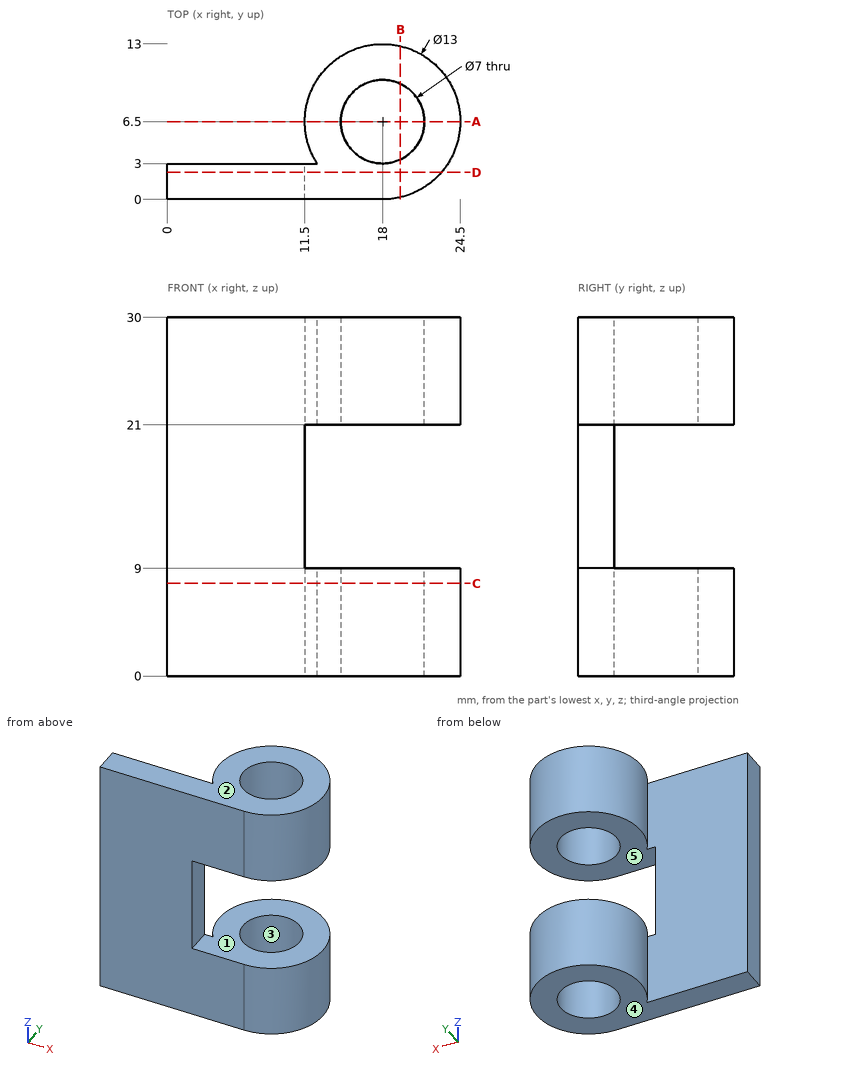
The figure shows three views and two pictorial views of one solid part (mm, origin at its lowest corner). Answer the questions. A direction names the side the tool comes from. Give positions to 0.01 mm unless a question says otherwise; leave off trailing zeros. Order: outer loops, then holes, each group sorted by start corner. A loop starts at its lowest first (then second) coordinate and runs counter-clockwise, first axis right, second up. Notation, with made-up numbers: (-13.5, -34) -> (13.5, -34) arc R27 ccw to (13.5, 0) -> close; hole circle Ø6 at (52.5, -6). An arc over 180 degrees is marked (long way). Answer as a JSON object with one key per item and string values. Group by question number.
Item 1: Determine the mould class of the marked faces 1, 2 and 3 for opening direction Z: pulls with the +Z half, pulls with the -Z half, needs draft (parallel to the pull), parting line crosses it, or undercut.
Item 2: The part is cut by section A-A on y = 6.5. Write down the section's boundary in (x, z), and give its area (3 significant figures).
Item 3: The part is cut by section C-C on z = 7.75. Write down the section's boundary in (x, y).
Item 4: Consider L1, parallel to X at y = 6.5, z = 4.25; L2, parallel to Z at x = 20.75, y = 2.75; L3, parallel to Y at x = 18, z = 7. Determine where each line is inside the solid, lowest interval first. Write a range as from..to.
Item 5: A tool of negligible diameter and unlimited length cuts with its end or side. For the marked faces 4 and 5, from which of +Z, -Z, +X, -X, +Y, -Y can it reach the whole face along a straight path? Write none if from no direction.
Item 6: Flat-ended cylindrical pins translate along their axes: pin 1 (6.5 mm diameter, centred on x = 18, y = 6.5, fed in from -Z); pin 2 (4 mm diameter, centred on x = 21, y = 8.5, fed in from -Z); pin 3 (12 mm diameter, centred on x = 4, z = 19.5, fed in from +Y); pin 4 (1.5 mm diameter, centred on y = 1.5, z = 18, fed in from +X). Find the tip coordinate at first contact, or state that the pin passes through.
Item 7: The part is cut by section B-B on x = 19.5. Write down the section's boundary in (y, z).
Item 8: The part is cut by section D-D on y = 2.25. Write down the section's boundary in (x, z).
Result set:
{
 "1": {"face 1": "undercut", "face 2": "pulls with the +Z half", "face 3": "needs draft"},
 "2": {"outline": "(11.5, 0) -> (14.5, 0) -> (14.5, 9) -> (11.5, 9) -> close; (11.5, 21) -> (14.5, 21) -> (14.5, 30) -> (11.5, 30) -> close; (21.5, 0) -> (24.5, 0) -> (24.5, 9) -> (21.5, 9) -> close; (21.5, 21) -> (24.5, 21) -> (24.5, 30) -> (21.5, 30) -> close", "area": "108 mm²"},
 "3": {"outline": "(0, 0) -> (18, 0) arc R6.5 ccw (long way) to (12.52, 3) -> (0, 3) -> close; hole circle Ø7 at (18, 6.5)"},
 "4": {"L1": "11.5..14.5, 21.5..24.5", "L2": "0..9, 21..30", "L3": "0..3, 10..13"},
 "5": {"face 4": "-Z, +X, -X, +Y, -Y", "face 5": "+X, +Y, -Y"},
 "6": {"pin 1": "through", "pin 2": "z = 0", "pin 3": "y = 3", "pin 4": "x = 11.5"},
 "7": {"outline": "(0.18, 0) -> (3.34, 0) -> (3.34, 9) -> (0.18, 9) -> close; (0.18, 21) -> (3.34, 21) -> (3.34, 30) -> (0.18, 30) -> close; (9.66, 0) -> (12.82, 0) -> (12.82, 9) -> (9.66, 9) -> close; (9.66, 21) -> (12.82, 21) -> (12.82, 30) -> (9.66, 30) -> close"},
 "8": {"outline": "(0, 0) -> (22.92, 0) -> (22.92, 9) -> (11.5, 9) -> (11.5, 21) -> (22.92, 21) -> (22.92, 30) -> (0, 30) -> close"}
}
